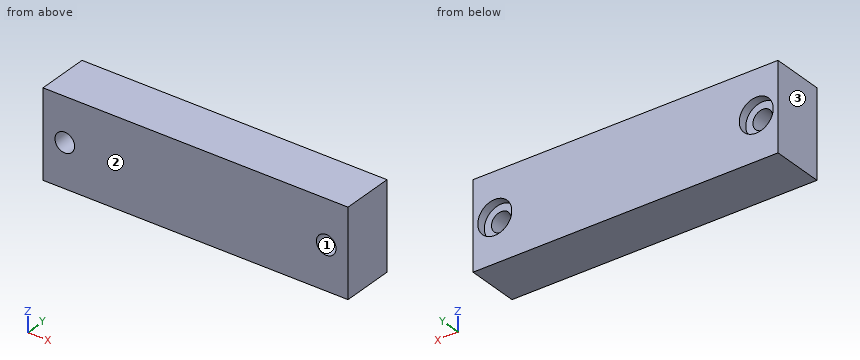
from build123d import *

# Parameters (mm, degrees)
SKETCH_1_W                = 70
SKETCH_1_H                = 20
EXTRUDE_1_DEPTH           = 12
HOLE_WIZARD_1_D           = 4.5
HOLE_WIZARD_1_CBORE_D     = 7.8
HOLE_WIZARD_1_CBORE_DEPTH = 2


with BuildPart() as part:
    # 草图1 → 凸台-拉伸1 (new body)
    with BuildSketch(Plane(origin=(0, 0, 0), x_dir=(1, 0, 0), z_dir=(0, 1, 0))):
        Rectangle(SKETCH_1_W, SKETCH_1_H)
    extrude(amount=EXTRUDE_1_DEPTH)

    # 打孔尺寸(%根据)内六角圆柱头螺钉的类型1 (through all)
    with Locations(Plane(origin=(0, 12, 0), x_dir=(1, 0, 0), z_dir=(0, 1, 0))):
        with Locations((-30, 0), (30, 0)):
            CounterBoreHole(HOLE_WIZARD_1_D / 2, HOLE_WIZARD_1_CBORE_D / 2, HOLE_WIZARD_1_CBORE_DEPTH)


solid = part.part
Could you check a few things on this model? Use its own coordinates, in mm. Face numbers are marked on the shaded views. Give positions to 0.01 mm unless a question says otherwise; leave off trailing zeros. Order: outer loops, then holes, each group sorted by start corner. A loop starts at its lowest first (then second) coordinate and runs counter-clockwise, first axis right, second up.
1. Suppose I cut it at D-D (y = 4.5). Write out the boundary of the cut face in (x, z), plus the area to 3 significant figures.
Answers below:
outline: (-35, -10) - (35, -10) - (35, 10) - (-35, 10) - close; hole circle Ø4.5 at (-30, 0); hole circle Ø4.5 at (30, 0)
area: 1,370 mm2
2. For pin 1 (6 mm diameter, centred on x = -30, z = 0, fed in from +Y); pin 2 (2.5 mm diameter, centred on x = 30, z = 0, fed in from +Y), each with a flat end and sliding along its axis, tell me the tip position at first contact or that it passes through.
Answers below:
pin 1: stops at y = 10
pin 2: passes through
3. Suppose I cut it at A-A (x = 30). Write out the boundary of the cut face in (y, z), plus the area to 3 significant figures.
Answers below:
outline: (0, -10) - (12, -10) - (12, -3.9) - (10, -3.9) - (10, -2.25) - (0, -2.25) - close; (0, 2.25) - (10, 2.25) - (10, 3.9) - (12, 3.9) - (12, 10) - (0, 10) - close
area: 179 mm2
4. Suppose I cut it at B-B (z = 1.5). Write out the boundary of the cut face in (x, y).
Answers below:
outline: (-35, 0) - (-31.68, 0) - (-31.68, 10) - (-33.6, 10) - (-33.6, 12) - (-35, 12) - close; (-28.32, 0) - (28.32, 0) - (28.32, 10) - (26.4, 10) - (26.4, 12) - (-26.4, 12) - (-26.4, 10) - (-28.32, 10) - close; (31.68, 0) - (35, 0) - (35, 12) - (33.6, 12) - (33.6, 10) - (31.68, 10) - close
5. Thinking about a two-plate mould opening in X: for the marked faces 1, 2 and 3, which applies, +X half, -X half, draft (parallel to the pull), parting line (faces both ways), or undercut?
Answers below:
face 1: undercut
face 2: draft
face 3: -X half
6. I need wall thicknesses on L1, parallel to X at y = 10.5, z = -1; L2, parallel to Z at x = -30, y = 10.8; L3, parallel to X at y = 4, z = -1.5. Which ranges of each line are inside material? Lowest first, please.
Answers below:
L1: x = -35 to -33.77, -26.23 to 26.23, 33.77 to 35
L2: z = -10 to -3.9, 3.9 to 10
L3: x = -35 to -31.68, -28.32 to 28.32, 31.68 to 35
7. Suppose I cut it at C-C (y = 11). Write out the boundary of the cut face in (x, z), plus the area to 3 significant figures.
Answers below:
outline: (-35, -10) - (35, -10) - (35, 10) - (-35, 10) - close; hole circle Ø7.8 at (-30, 0); hole circle Ø7.8 at (30, 0)
area: 1,300 mm2
